Read the model definition and answer for the solid it produces. Units are mm, in the model's axes. A direction names the side the tool comes from. Round coordinates to 2 decimals unless told otherwise and drop trailing zeros. Write each loop counter-clockwise with the first axis right and the second up, starting at its lowest first coordinate (ties: lowest second). Pieces come first, ordered by that corner, then holes. Notation, with made-up numbers: (5.5, -35) -> (33.5, -35) arc R20 ccw to (33.5, 3) -> close; hole circle Ø3 at (-26.75, -2.75). An arc over 180 degrees is marked (long way). Return JSON: item names as keys, results as strings.
from build123d import *

# Parameters (mm, degrees)
FRONT_RING_PROFILE_110_R  = 55
FRONT_RING_DISC_DEPTH     = 10
REAR_RING_PROFILE_R       = 55
REAR_RING_DISC_DEPTH      = 10
RING_BORE_90_PROFILE_R    = 45
RING_BORE_90_DEPTH        = 105.642247682
FRONT_CLAMP_BRACKET_DEPTH = 10
REAR_CLAMP_BRACKET_DEPTH  = 10
CAGE_RODS_6X_10_PROFILE_R = 5
CAGE_RODS_6X_10_DEPTH     = 50


with BuildPart() as part:
    # Front Ring Profile Ø110 → Front Ring Disc (new body)
    with BuildSketch(Plane.XY):
        Circle(FRONT_RING_PROFILE_110_R)
    extrude(amount=-FRONT_RING_DISC_DEPTH)


with BuildPart() as body_2:
    # Rear Ring Profile → Rear Ring Disc (new body)
    with BuildSketch(Plane.XY.offset(-70)):
        Circle(REAR_RING_PROFILE_R)
    extrude(amount=REAR_RING_DISC_DEPTH)


with BuildPart() as ring_bore_90_tool:
    # Ring Bore Ø90 Profile → Ring Bore Ø90 (new, through all)
    with BuildSketch(Plane.XY):
        Circle(RING_BORE_90_PROFILE_R)
    extrude(amount=-RING_BORE_90_DEPTH)


with BuildPart() as part_1:
    add(part.part)

    # Ring Bore Ø90: cut by ring_bore_90_tool
    add(ring_bore_90_tool.part, mode=Mode.SUBTRACT)



with BuildPart() as body_2_1:
    add(body_2.part)

    # Ring Bore Ø90: cut by ring_bore_90_tool
    add(ring_bore_90_tool.part, mode=Mode.SUBTRACT)


with BuildPart() as part_2:
    add(part_1.part)

    add(body_2_1.part)  # Front Clamp Bracket merges body 2
    # Front Clamp Bracket Profile → Front Clamp Bracket (add)
    with BuildSketch(Plane(origin=(20, 0, 0), x_dir=(0, 0, -1), z_dir=(1, 0, 0))):
        Polygon((0, 45), (0, 90), (70, 90), (70, 45), (60, 45), (60, 80), (10, 80), (10, 45), align=None)
    extrude(amount=-FRONT_CLAMP_BRACKET_DEPTH)

    # Rear Clamp Bracket Profile → Rear Clamp Bracket (add)
    with BuildSketch(Plane(origin=(-20, 0, 0), x_dir=(0, 0, -1), z_dir=(1, 0, 0))):
        Polygon((10, 80), (60, 80), (60, 51.23475383), (70, 51.23475383), (70, 90), (0, 90), (0, 51.23475383), (10, 51.23475383), align=None)
    extrude(amount=REAR_CLAMP_BRACKET_DEPTH)

    # Cage Rods 6xØ10 Profile → Cage Rods 6xØ10 (add)
    with BuildSketch(Plane(origin=(0, 0, -10), x_dir=(-1, 0, 0), z_dir=(0, 0, -1))):
        with Locations(Location((50, 0, 0), (0, 0, 180))):
            Circle(CAGE_RODS_6X_10_PROFILE_R)
        with Locations(Location((25, -43.301270189, 0), (0, 0, 120))):
            Circle(CAGE_RODS_6X_10_PROFILE_R)
        with Locations(Location((-25, -43.301270189, 0), (0, 0, 240))):
            Circle(CAGE_RODS_6X_10_PROFILE_R)
        with Locations(Location((-50, 0, 0), (0, 0, 180))):
            Circle(CAGE_RODS_6X_10_PROFILE_R)
        with Locations(Location((-25, 43.301270189, 0), (0, 0, 120))):
            Circle(CAGE_RODS_6X_10_PROFILE_R)
        with Locations(Location((25, 43.301270189, 0), (0, 0, 240))):
            Circle(CAGE_RODS_6X_10_PROFILE_R)
    extrude(amount=CAGE_RODS_6X_10_DEPTH)


solid = part_2.part
Item 1: Section C-C (y = 21.5) is taken. Give the vertices of the cut face in (x, z), then the cut area to 3 significant figures.
Worked answers:
{"outline": "(-50.62, -70) -> (-39.53, -70) -> (-39.53, -60) -> (-50.62, -60) -> close; (-50.62, -10) -> (-39.53, -10) -> (-39.53, 0) -> (-50.62, 0) -> close; (39.53, -70) -> (50.62, -70) -> (50.62, -60) -> (39.53, -60) -> close; (39.53, -10) -> (50.62, -10) -> (50.62, 0) -> (39.53, 0) -> close", "area": "444 mm2"}
Item 2: Section B-B (z = -36.5) is taken. Give the vertices of the cut face in (x, y).
Worked answers:
{"outline": "circle Ø10 at (-50, 0); circle Ø10 at (-25, -43.3); circle Ø10 at (-25, 43.3); (-20, 80) -> (-10, 80) -> (-10, 90) -> (-20, 90) -> close; (10, 80) -> (20, 80) -> (20, 90) -> (10, 90) -> close; circle Ø10 at (25, -43.3); circle Ø10 at (25, 43.3); circle Ø10 at (50, 0)"}
Item 3: Straight lines are drawn through the part: L1, parallel to Y at x = 0, z = -63; L2, parallel to X at y = 0.5, z = -35; L3, parallel to X at y = 54, z = -8.5. For each, find the intervals that lie inside material, in ascending order. Write a range as [from, to].
Worked answers:
{"L1": "y = [-55, -45], [45, 55]", "L2": "x = [-54.97, -45.03], [45.03, 54.97]", "L3": "x = [-20, 20]"}
Item 4: A tool of negligible diameter and unlimited length cuts with its end or side. For faces 1 (the cylindrical face through (20.765, -39.923, -64.93)), 2 (the flat face through (15, 80, -35)), from which of +Z, -Z, +X, -X, +Y, -Y can it reach the whole face along a straight path? Write none if from no direction.
Worked answers:
{"face 1": "+Z, -Z", "face 2": "+X, -X, -Y"}
Item 5: For a pull along Y with two mould halves and no side action, classify faces 3 (the cylindrical face through (-21.315, 46.681, -34.65)), 4 (the flat face through (10, 80.3, -35.5)), 5 (the cylindrical face through (45, 0, -35)) as released by +Y, released by -Y, zero draft, split by the parting line, or undercut.
Worked answers:
{"face 3": "undercut", "face 4": "zero draft", "face 5": "split by the parting line"}
Item 6: Section D-D (x = 12.5) is taken. Give the vertices of the cut face in (y, z).
Worked answers:
{"outline": "(-53.56, -70) -> (-43.23, -70) -> (-43.23, -60) -> (-53.56, -60) -> close; (-53.56, -10) -> (-43.23, -10) -> (-43.23, 0) -> (-53.56, 0) -> close; (43.23, -70) -> (90, -70) -> (90, 0) -> (43.23, 0) -> (43.23, -10) -> (80, -10) -> (80, -60) -> (43.23, -60) -> close"}
Item 7: Section A-A (x = 0) is taken. Give the vertices of the cut face in (y, z), then the cut area to 3 significant figures.
Worked answers:
{"outline": "(-55, -70) -> (-45, -70) -> (-45, -60) -> (-55, -60) -> close; (-55, -10) -> (-45, -10) -> (-45, 0) -> (-55, 0) -> close; (45, -70) -> (55, -70) -> (55, -60) -> (45, -60) -> close; (45, -10) -> (55, -10) -> (55, 0) -> (45, 0) -> close", "area": "400 mm2"}
Item 8: Flat-ended cylindrical pins translate along their axes: pin 1 (8 mm diameter, centred on x = -25, z = -54, fed in from -Y); pin 2 (5 mm diameter, centred on x = 13.5, z = -38.5, fed in from -Y); pin 3 (11 mm diameter, centred on x = -15.5, z = -39, fed in from -Y). Find the tip coordinate at first contact, or state that the pin passes through.
Worked answers:
{"pin 1": "stops at y = -48.3", "pin 2": "stops at y = 80", "pin 3": "stops at y = -46.3"}
